from build123d import *

# Parameters (mm, degrees)
SKETCH1_R           = 1.75
BOSS_EXTRUDE1_DEPTH = 4.25
SKETCH2_R           = 3
BOSS_EXTRUDE2_DEPTH = 4.25
SKETCH3_R           = 2.75
BOSS_EXTRUDE3_DEPTH = 0.5
SKETCH4_R           = 3
BOSS_EXTRUDE4_DEPTH = 2.5
SKETCH5_R           = 3.25
BOSS_EXTRUDE5_DEPTH = 5
SKETCH6_R           = 4.25
BOSS_EXTRUDE6_DEPTH = 10
CHAMFER1_SIZE       = 0.5
CHAMFER1_SIZE2      = 4
SKETCH7_R           = 4.7
BOSS_EXTRUDE7_DEPTH = 8
SKETCH8_R           = 2
BOSS_EXTRUDE8_DEPTH = 2.5
FILLET1_R           = 2


with BuildPart() as part:
    # Sketch1 → Boss-Extrude1 (new body)
    with BuildSketch(Plane(origin=(0, 0, 0), x_dir=(1, 0, 0), z_dir=(0, 1, 0))):
        with Locations(Location((0, 0, 0), (0, 0, 270))):
            Circle(SKETCH1_R)
    extrude(amount=BOSS_EXTRUDE1_DEPTH)

    # Sketch2 → Boss-Extrude2 (add)
    with BuildSketch(Plane(origin=(0, 4.25, 0), x_dir=(1, 0, 0), z_dir=(0, 1, 0))):
        with Locations(Location((0, 0, 0), (0, 0, 270))):
            Circle(SKETCH2_R)
    extrude(amount=BOSS_EXTRUDE2_DEPTH)

    # Sketch3 → Boss-Extrude3 (add)
    with BuildSketch(Plane(origin=(0, 8.5, 0), x_dir=(1, 0, 0), z_dir=(0, 1, 0))):
        with Locations(Location((0, 0, 0), (0, 0, 270))):
            Circle(SKETCH3_R)
    extrude(amount=BOSS_EXTRUDE3_DEPTH)

    # Sketch4 → Boss-Extrude4 (add)
    with BuildSketch(Plane(origin=(0, 9, 0), x_dir=(1, 0, 0), z_dir=(0, 1, 0))):
        with Locations(Location((0, 0, 0), (0, 0, 270))):
            Circle(SKETCH4_R)
    extrude(amount=BOSS_EXTRUDE4_DEPTH)

    # Sketch5 → Boss-Extrude5 (add)
    with BuildSketch(Plane(origin=(0, 11.5, 0), x_dir=(1, 0, 0), z_dir=(0, 1, 0))):
        with Locations(Location((0, 0, 0), (0, 0, 270))):
            Circle(SKETCH5_R)
    extrude(amount=BOSS_EXTRUDE5_DEPTH)

    # Sketch6 → Boss-Extrude6 (add)
    with BuildSketch(Plane(origin=(0, 16.5, 0), x_dir=(1, 0, 0), z_dir=(0, 1, 0))):
        with Locations(Location((0, 0, 0), (0, 0, 270))):
            Circle(SKETCH6_R)
    extrude(amount=BOSS_EXTRUDE6_DEPTH)

    # Chamfer1
    chamfer1_edges = [part.edges().sort_by_distance(p)[0] for p in [
        (0, 16.5, -4.25),
    ]]
    chamfer1_side = [part.faces().sort_by_distance(p)[0] for p in [
        (0, 16.5, -4.129791847),
    ]]
    chamfer(chamfer1_edges, length=CHAMFER1_SIZE, length2=CHAMFER1_SIZE2, reference=chamfer1_side[0])

    # Sketch7 → Boss-Extrude7 (add)
    with BuildSketch(Plane(origin=(0, 26.5, 0), x_dir=(1, 0, 0), z_dir=(0, 1, 0))):
        with Locations(Location((0, 0, 0), (0, 0, 270))):
            Circle(SKETCH7_R)
    extrude(amount=BOSS_EXTRUDE7_DEPTH)

    # Sketch8 → Boss-Extrude8 (add)
    with BuildSketch(Plane(origin=(0, 34.5, 0), x_dir=(1, 0, 0), z_dir=(0, 1, 0))):
        with Locations(Location((0, 0, 0), (0, 0, 270))):
            Circle(SKETCH8_R)
    extrude(amount=BOSS_EXTRUDE8_DEPTH)

    # Fillet1
    fillet1_edges = [part.edges().sort_by_distance(p)[0] for p in [
        (0, 37, -2),
    ]]
    fillet(fillet1_edges, radius=FILLET1_R)


solid = part.part
Can you work these out from the model? Positions are in its coordinate system, mm. A direction names the side the tool comes from. Give positions to 0.01 mm unless a question says otherwise; leave off trailing zeros. Order: outer loops, then holes, each group sorted by start corner. A loop starts at its lowest first (then second) coordinate and runs counter-clockwise, first axis right, second up. Notation, with made-up numbers: M 75.5,64 L 109.5,64 A20 ccw 109.5,88 Z; hole C 28.25,10 d4. An arc over 180 degrees is marked long. Use a Markdown table: item, result. Add a question column.
Item 1: Suppose I cut it at C-C (y = 6.5). List the corners of the cut face in (x, z) for me, then the cut area to 3 significant figures.
Item 2: Suppose I cut it at D-D (y = 24). List the corners of the cut face in (x, z) for me, then the cut area to 3 significant figures.
Item 3: We'd pull the mould along Y, two halves only. Please class faces 4 (the cylindrical face through (-2.685, 8.746, -0.596)), 5 (the cylindrical face through (0.9, 6.35, 2.86)), 6 (the flat face through (-2, 34.5, 1)), 7 (the flat face through (-2, 26.5, -4)): +Y half, -Y half, draft (parallel to the pull), parting line (faces both ways), or undercut.
Item 4: For faces 1 (the cylindrical face through (4.214, 23.458, -0.553)), 2 (the cylindrical face through (-1.952, 34.746, -0.434)), 3 (the flat face through (0, 0, 0)), which set-ups out of +Z, -Z, +X, -X, +Y, -Y let a thin tool reach every point of the face, with its end or its side?
Item 5: If I drill on L1, parallel to Y at x = 0.75, z = 4.25; L2, parallel to Z at x = 2, y = 27; L3, parallel to Y at x = -2, z = 2.5, over which ranges is the centre line in solid material (lowest first)? Write a range as [from, to].
Item 6: Will these pins go through, and if not, where does the flat tip stop? pin 1 (1 mm diameter, centred on x = 1, y = 12, fed in from +Z); pin 2 (3 mm diameter, centred on x = 1, z = 1.5, fed in from -Y); pin 3 (5 mm diameter, centred on x = 1.5, z = 2.5, fed in from +Y); pin 4 (1.5 mm diameter, centred on y = 17, z = -3, fed in from -X).
Answer sheet:
| question | item | result |
|---|---|---|
| 1 | outline | C 0,0 d6 |
| 1 | area | 28.3 mm² |
| 2 | outline | C 0,0 d8.5 |
| 2 | area | 56.7 mm² |
| 3 | face 4 | undercut |
| 3 | face 5 | draft |
| 3 | face 6 | +Y half |
| 3 | face 7 | -Y half |
| 4 | face 1 | -Y |
| 4 | face 2 | +Y |
| 4 | face 3 | +Z, -Z, +X, -X, -Y |
| 5 | L1 | y = [26.5, 34.5] |
| 5 | L2 | z = [-4.25, 4.25] |
| 5 | L3 | y = [11.5, 34.5] |
| 6 | pin 1 | stops at z = 3.21 |
| 6 | pin 2 | stops at y = 0 |
| 6 | pin 3 | stops at y = 36.96 |
| 6 | pin 4 | stops at x = -3.09 |
